from build123d import *

# Parameters (mm, degrees)
SKETCH1_W               = 50
SKETCH1_H               = 50
BOSS_EXTRUDE1_DEPTH     = 500
SKETCH2_W               = 50
SKETCH2_H               = 50
BOSS_EXTRUDE2_DEPTH     = 450
SKETCH3_W               = 50
SKETCH3_H               = 50
BOSS_EXTRUDE3_DEPTH     = 1750
SKETCH4_W               = 50
SKETCH4_H               = 50
BOSS_EXTRUDE4_DEPTH     = 450
SKETCH5_W               = 50
SKETCH5_H               = 50
BOSS_EXTRUDE5_DEPTH     = 400
CUT_EXTRUDE1_REACH      = 1912.661
SKETCH6_R               = 10
LPATTERN1_COUNT         = 6
LPATTERN1_PITCH         = 300
SKETCH8_R               = 8
CUT_EXTRUDE2_DEPTH      = 1928.59565262
SKETCH9_W               = 15
SKETCH9_H               = 40
BOSS_EXTRUDE6_DEPTH     = 30
SKETCH12_W              = 15
SKETCH12_H              = 40
BOSS_EXTRUDE7_DEPTH     = 30
SKETCH13_W              = 15
SKETCH13_H              = 40
BOSS_EXTRUDE8_DEPTH     = 48
CUT_EXTRUDE3_DEPTH      = 1913.367642479
CUT_EXTRUDE3_DEPTH_BACK = 1913.367642479
SKETCH14_R              = 7.5
SKETCH15_R              = 7.5
SKETCH15_R_2            = 5.5
BOSS_EXTRUDE9_DEPTH     = 15


with BuildPart() as part:
    # Sketch1 → Boss-Extrude1 (new body)
    with BuildSketch(Plane.XY):
        Rectangle(SKETCH1_W, SKETCH1_H)
    extrude(amount=BOSS_EXTRUDE1_DEPTH)

    # Sketch2 → Boss-Extrude2 (add)
    with BuildSketch(Plane(origin=(0, 25, 0), x_dir=(1, 0, 0), z_dir=(0, 1, 0))):
        with Locations((0, -25)):
            Rectangle(SKETCH2_W, SKETCH2_H)
        with Locations((0, -475)):
            Rectangle(SKETCH2_W, SKETCH2_H)
    extrude(amount=BOSS_EXTRUDE2_DEPTH)

    # Sketch3 → Boss-Extrude3 (add)
    with BuildSketch(Plane(origin=(25, 0, 0), x_dir=(0, 0, -1), z_dir=(1, 0, 0))):
        with Locations((-475, 450)):
            Rectangle(SKETCH3_W, SKETCH3_H)
        with Locations((-25, 450)):
            Rectangle(SKETCH3_W, SKETCH3_H)
    extrude(amount=BOSS_EXTRUDE3_DEPTH)

    # Sketch4 → Boss-Extrude4 (add)
    with BuildSketch(Plane(origin=(0, 425, 0), x_dir=(-1, 0, 0), z_dir=(0, -1, 0))):
        with Locations((-1750, -475)):
            Rectangle(SKETCH4_W, SKETCH4_H)
        with Locations((-1750, -25)):
            Rectangle(SKETCH4_W, SKETCH4_H)
    extrude(amount=BOSS_EXTRUDE4_DEPTH)

    # Sketch5 → Boss-Extrude5 (add)
    with BuildSketch(Plane(origin=(0, 0, 450), x_dir=(-1, 0, 0), z_dir=(0, 0, -1))):
        with Locations((-1750, 0)):
            Rectangle(SKETCH5_W, SKETCH5_H)
    extrude(amount=BOSS_EXTRUDE5_DEPTH)

    # Sketch6 → Cut-Extrude1 (cut, up to next)
    with BuildSketch(Plane(origin=(0, 475, 0), x_dir=(1, 0, 0), z_dir=(0, 1, 0)), mode=Mode.PRIVATE) as cut_extrude1_sk1:
        with Locations(Location((125, -25, 0), (0, 0, 270))):
            Circle(SKETCH6_R)
    cut_extrude1_tool1 = extrude(cut_extrude1_sk1.sketch, amount=-CUT_EXTRUDE1_REACH, mode=Mode.PRIVATE) & part.part
    # Sketch6 → Cut-Extrude1 (cut, up to next)
    with BuildSketch(Plane(origin=(0, 475, 0), x_dir=(1, 0, 0), z_dir=(0, 1, 0)), mode=Mode.PRIVATE) as cut_extrude1_sk2:
        with Locations(Location((125, -475, 0), (0, 0, 270))):
            Circle(SKETCH6_R)
    cut_extrude1_tool2 = extrude(cut_extrude1_sk2.sketch, amount=-CUT_EXTRUDE1_REACH, mode=Mode.PRIVATE) & part.part
    cut_extrude1_1 = cut_extrude1_tool1.solids().sort_by_distance((125, 475, 25))[0]
    add(cut_extrude1_1, mode=Mode.SUBTRACT)
    cut_extrude1_2 = cut_extrude1_tool2.solids().sort_by_distance((125, 475, 475))[0]
    add(cut_extrude1_2, mode=Mode.SUBTRACT)
    cut_extrude1 = cut_extrude1_1 + cut_extrude1_2  # Cut-Extrude1 as one shape, for the pattern or mirror that repeats it

    # LPattern1: Cut-Extrude1 ×6
    with Locations(*[(i * LPATTERN1_PITCH, 0, 0) for i in range(1, LPATTERN1_COUNT)]):
        add(cut_extrude1, mode=Mode.SUBTRACT)

    # Sketch8 → Cut-Extrude2 (cut, through all)
    with BuildSketch(Plane.ZY.offset(25)):
        with Locations((475, 95)):
            Circle(SKETCH8_R)
        with Locations((25, 95)):
            Circle(SKETCH8_R)
    extrude(amount=-CUT_EXTRUDE2_DEPTH, mode=Mode.SUBTRACT)

    # Sketch9 → Boss-Extrude6 (add)
    with BuildSketch(Plane(origin=(0, 0, 450), x_dir=(-1, 0, 0), z_dir=(0, 0, -1))):
        with Locations((17.5, 95)):
            Rectangle(SKETCH9_W, SKETCH9_H)
    extrude(amount=BOSS_EXTRUDE6_DEPTH)

    # Sketch12 → Boss-Extrude7 (add)
    with BuildSketch(Plane(origin=(0, 0, 0), x_dir=(-1, 0, 0), z_dir=(0, 0, -1))):
        with Locations((17.5, 95)):
            Rectangle(SKETCH12_W, SKETCH12_H)
    extrude(amount=BOSS_EXTRUDE7_DEPTH)

    # Sketch13 → Boss-Extrude8 (add)
    with BuildSketch(Plane.ZY.offset(25)):
        with Locations((-22.5, 95)):
            Rectangle(SKETCH13_W, SKETCH13_H)
        with Locations((427.5, 95)):
            Rectangle(SKETCH13_W, SKETCH13_H)
    extrude(amount=BOSS_EXTRUDE8_DEPTH)

    # Sketch14 → Cut-Extrude3 (cut, two sides: drawn at the far end of the back side and taken through both)
    with BuildSketch(Plane(origin=(0, 0, -30), x_dir=(-1, 0, 0), z_dir=(0, 0, -1)).offset(-CUT_EXTRUDE3_DEPTH_BACK)):
        with Locations(Location((53, 95, 0), (0, 0, 90))):
            Circle(SKETCH14_R)
    extrude(amount=CUT_EXTRUDE3_DEPTH + CUT_EXTRUDE3_DEPTH_BACK, mode=Mode.SUBTRACT)

    # Sketch15 → Boss-Extrude9 (add)
    with BuildSketch(Plane(origin=(0, 0, -30), x_dir=(-1, 0, 0), z_dir=(0, 0, -1))):
        with Locations((53, 95)):
            Circle(SKETCH15_R)
        with Locations((53, 95)):
            Circle(SKETCH15_R_2, mode=Mode.SUBTRACT)
    extrude(amount=-BOSS_EXTRUDE9_DEPTH)


solid = part.part
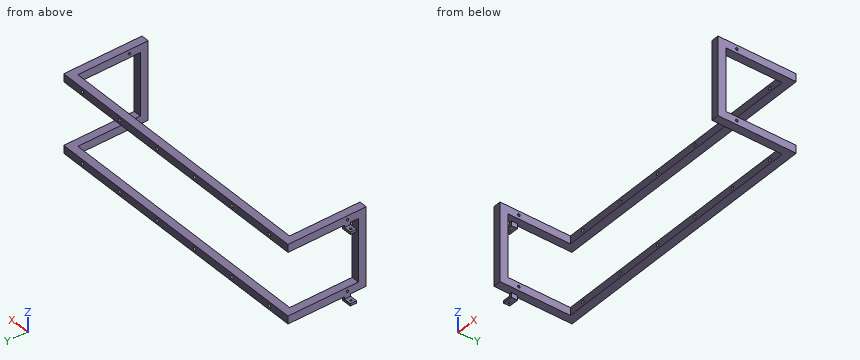
The model under review builds one solid part; all positions refer to its coordinate system, in mm. Give positions to 0.01 mm unless a question says otherwise; leave off trailing zeros. Loops run counter-clockwise (first coordinate to the right, second up) from the corner with the lowest first, then second, coordinate; pieces in that order, holes last. Notation, with made-up numbers: (-31.75, 45) -> (-1.75, 45) arc R23 ccw to (-1.75, 71) -> close; hole circle Ø3 at (-12, 48.5). An arc over 180 degrees is marked (long way). Answer as a JSON object with one key per item and string values. Group by question number.
Q1. Take a section at C-C (y = 367). Write out the cut boundary in (x, z).
Q2. Insertion check: pin 1 (9 mm diameter, centred on x = -47.5, z = 430.5, fed in from +Y); pin 2 (9 mm diameter, centred on x = -43.5, z = -20.5, fed in from -Y). Each pin has a flat end and moves straight along its axis. Give the tip position at first contact, or say it passes through.
Q3. Take a section at B-B (x = 491.5). Write out the cut boundary in (y, z), plus the area to 3 significant figures.
Q4. Wall thickness on line 1 along Y through (x, z) = (-53, -20.5); line 2 along X through (y, z) = (142.5, 475.5); line 3 along Y through (x, z) = (1764, 25): over which ranges is each line inside the solid? List them lowest first.
Q5. Take a section at A-A (z = 127.5). Write out the cut boundary in (x, y).
Answer below:
{
 "1": {"outline": "(-25, 0) -> (25, 0) -> (25, 50) -> (-25, 50) -> close; (-25, 450) -> (25, 450) -> (25, 500) -> (-25, 500) -> close; (1725, 0) -> (1775, 0) -> (1775, 50) -> (1725, 50) -> close; (1725, 450) -> (1775, 450) -> (1775, 500) -> (1725, 500) -> close"},
 "2": {"pin 1": "stops at y = 115", "pin 2": "stops at y = 75"},
 "3": {"outline": "(425, 0) -> (475, 0) -> (475, 50) -> (425, 50) -> close; (425, 450) -> (475, 450) -> (475, 500) -> (425, 500) -> close", "area": "5,000 mm2"},
 "4": {"line 1": "y = 75 to 89.5, 100.5 to 115", "line 2": "x = -25 to 25, 1725 to 1775", "line 3": "y = -25 to 87, 103 to 475"},
 "5": {"outline": "(-25, -25) -> (25, -25) -> (25, 25) -> (-25, 25) -> close; (1725, -25) -> (1775, -25) -> (1775, 25) -> (1725, 25) -> close"}
}
